Verification items for the finished model (mm, model axes). Face numbers are marked on the shaded views. A direction names the side the tool comes from. Coordinates: 2 decimals unless noted, no trailing zeros. Write each loop counter-clockwise with the first axis right and the second up, starting at its lowest first coordinate (ties: lowest second). Pieces come first, ordered by that corner, then holes. Notation, with made-up numbers: (40, 49) - (89, 49) arc R22 ccw to (89, 78) - close; hole circle Ø3 at (-27.5, -30). An arc over 180 degrees is marked (long way). Use one line per item in the form item = value. Start each with the question number.
(1) Sectioned sample at A-A (z = 0). Record the cut outline in (x, y).
(2) Material ranges on line 1 (Z direction, x = 11.5, y = -0.5); line 2 (X direction, y = -0.5, z = 7.5); line 3 (X direction, y = -7, z = 13.5), recorded low to high. Write a range as [from, to].
(3) Sectioned sample at D-D (x = 10). Record the cut outline in (y, z).
(4) Gauge pin test, flat ends, axial feed: pin 1 Ø10 at (x, z) = (8.5, 9.5) entering from -Y; pin 2 Ø8 at (x, z) = (14, 4) entering from +Y; pin 3 Ø1.5 at (x, y) = (15, -0.5) entering from -Z. Record the tip position at first contact, or that the pin passes through.
(5) Sectioned sample at C-C (x = 3). Record the cut outline in (y, z), and give its area (3 significant figures).
(6) Tool access check on the marked faces 1 and 2. Record the directions out of +Z, -Z, +X, -X, +Y, -Y that give a thin tool (end or side, any length) a straight path to the whole face; none if there is none.
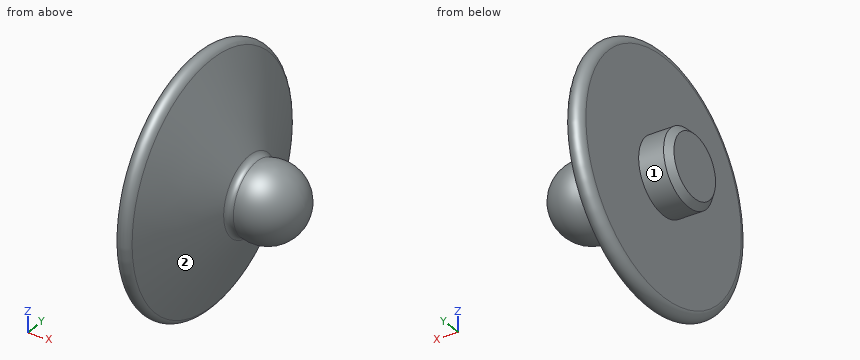
from build123d import *

# Parameters (mm, degrees)
CHAMFER1_SIZE = 1


with BuildPart() as part:
    # Sketch1 → Revolve1 (revolve)
    with BuildSketch(Plane.XY, mode=Mode.PRIVATE) as revolve1_sk:
        with BuildLine():
            Line((0, 0), (0, 6))
            Line((0, 6), (5, 6))
            Line((5, 6), (5, 18.672111461))
            ThreePointArc((5, 18.672111461), (6.040480856, 19.96852374), (7.531364262, 19.233301407))
            Line((7.531364262, 19.233301407), (13.572014794, 6.279084538))
            ThreePointArc((13.572014794, 6.279084538), (14.069886887, 5.788915703), (14.767133641, 5.744316685))
            ThreePointArc((14.767133641, 5.744316685), (20.077904543, 4.816492404), (22.5, 0))
            Line((22.5, 0), (0, 0))
        make_face()
    revolve(revolve1_sk.sketch.rotate(Axis((0, 0, 0), (1, 0, 0)), 90), axis=Axis((0, 0, 0), (1, 0, 0)))

    # Chamfer1
    chamfer1_edges = [part.edges().sort_by_distance(p)[0] for p in [
        (0, 0, -6),
    ]]
    chamfer(chamfer1_edges, length=CHAMFER1_SIZE)


solid = part.part
Answers below:
q1.outline = (0, -5) - (1, -6) - (5, -6) - (5, -18.67) arc R1.33 ccw to (7.53, -19.23) - (13.57, -6.28) arc R1 cw to (14.77, -5.74) arc R6 ccw (long way) to (14.77, 5.74) arc R1 cw to (13.57, 6.28) - (7.53, 19.23) arc R1.33 ccw to (5, 18.67) - (5, 6) - (1, 6) - (0, 5) - close
q2.line_1 = [-10.71, 10.71]
q2.line_2 = [5, 12.99]
q2.line_3 = [5, 9.41]
q3.outline = circle Ø27.88 at (0, 0)
q4.pin_1 = -19.37
q4.pin_2 = 13.42
q4.pin_3 = -5.94
q5.outline = circle Ø12 at (0, 0)
q5.area = 113 mm2
q6.face_1 = -X
q6.face_2 = +X
